Design review of the part built by this model. Coordinates are the model's own, in mm. Face numbers are marked on the shaded views. A direction names the side the tool comes from. Round coordinates to 2 decimals unless told otherwise and drop trailing zeros. Loops run counter-clockwise (first coordinate to the right, second up) from the corner with the lowest first, then second, coordinate; pieces in that order, holes last. Notation, with made-up numbers: M -32,35 L 5,35 A33 cw 5,63 Z; hole C -11.5,-33.75 d8. An arc over 180 degrees is marked long. One line per item, written item: value. Start each with the question number.
Item 1: Clearance check with flat-ended pins moving along their axes: pin 1 (1.5 mm diameter, centred on y = -1.5, z = -57.5, fed in from +X); pin 2 (1.5 mm diameter, centred on x = 2.5, y = -1.5, fed in from +Z); pin 3 (3 mm diameter, centred on y = -1.5, z = -32.5, fed in from -X). State where each tip first meets the part, or that it passes through.
Item 2: We need section A-A (y = 0). Write out the cut boundary in (x, z), then the cut area to 3 significant figures.
Item 3: For the marked faces 1, 2 and 3, list the 3-axis set-ups (+Z, -Z, +X, -X, +Y, -Y) from which the entire face can be reached by the end or side of a thin tool; tool diameter is ignored.
Item 4: For line 1 along Y through (x, z) = (-0.25, -35); line 2 along Z through (x, y) = (-1, 3.5); line 3 along X through (y, z) = (2.75, -46.5), list the stretches that pass through material, from the lowest coordinate up.
Item 5: We need section C-C (z = -53.5). Write out the cut boundary in (x, y).
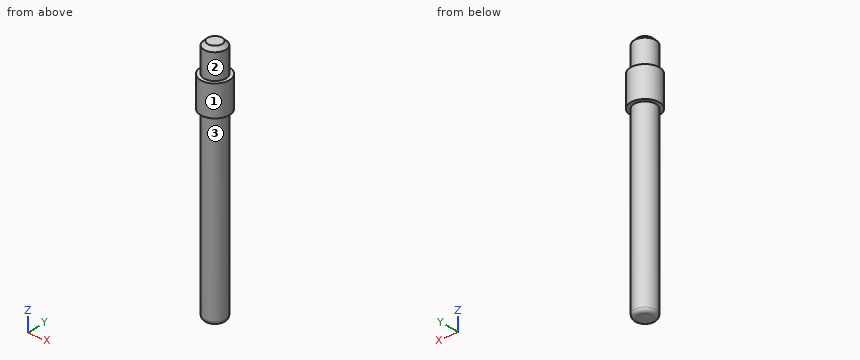
from build123d import *

# Parameters (mm, degrees)
FILLET_1_R     = 1
CHAMFER_1_SIZE = 1


with BuildPart() as part:
    # 草图1 → 旋转1 (revolve)
    with BuildSketch(Plane(origin=(0, 0, 0), x_dir=(0, 0, -1), z_dir=(1, 0, 0))):
        Polygon((0, 0), (0, 3), (8, 3), (8, 4), (16.5, 4), (16.5, 3), (67.5, 3), (67.5, 0), align=None)
    revolve(axis=Axis((0, 0, -67.5), (0, 0, 1)))

    # 圆角1
    fillet_1_edges = [part.edges().sort_by_distance(p)[0] for p in [
        (0, -3, -67.5),
    ]]
    fillet(fillet_1_edges, radius=FILLET_1_R)

    # 倒角1
    chamfer_1_edges = [part.edges().sort_by_distance(p)[0] for p in [
        (0, -3, 0),
    ]]
    chamfer(chamfer_1_edges, length=CHAMFER_1_SIZE)


solid = part.part
A:
1. pin 1: x = 2.9
1. pin 2: z = -0.17
1. pin 3: x = -3
2. outline: M -4,-16.5 L -3,-16.5 L -3,-66.5 A1 ccw -2,-67.5 L 2,-67.5 A1 ccw 3,-66.5 L 3,-16.5 L 4,-16.5 L 4,-8 L 3,-8 L 3,-1 L 2,0 L -2,0 L -3,-1 L -3,-8 L -4,-8 Z
2. area: 421 mm2
3. face 1: +Z, -Z
3. face 2: +Z
3. face 3: -Z
4. line 1: -2.99 to 2.99
4. line 2: -16.5 to -8
4. line 3: -1.2 to 1.2
5. outline: C 0,0 d6
